Here's the drawing with two shaded views (mm, measured from the low corner). I have some questions. Coordinates: 2 decimals unless noted, no trailing zeros. Loops run counter-clockwise (first coordinate to the right, second up) from the corner with the lowest first, then second, coordinate; pieces in that order, holes last.
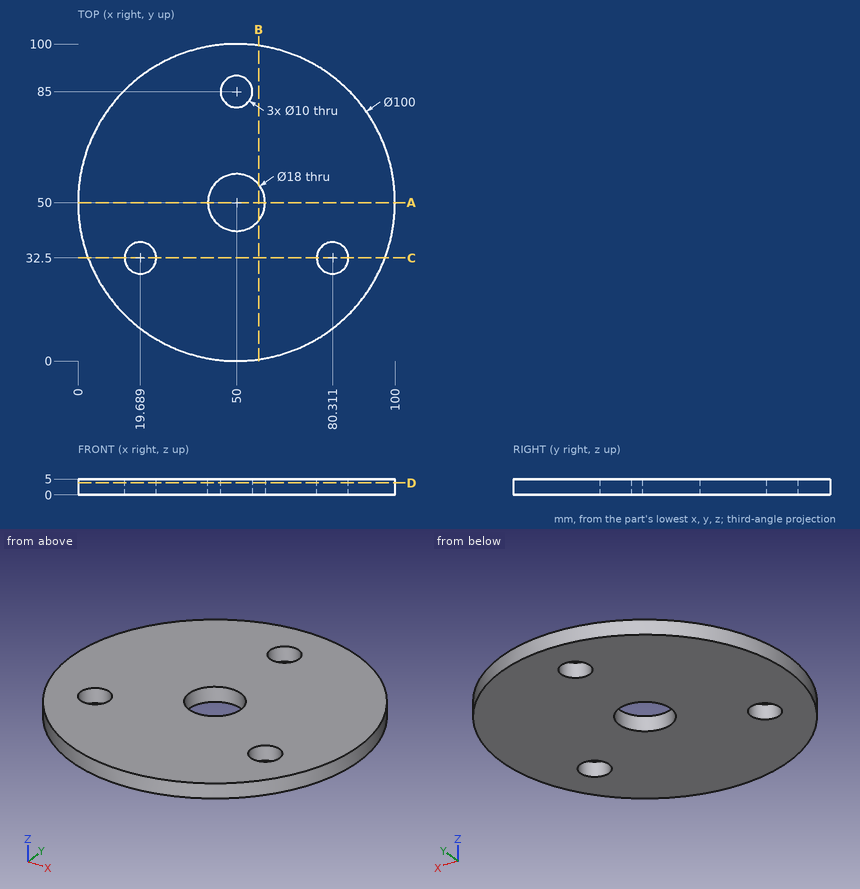
Q1. Suppose I cut it at B-B on x = 57. Write out the boundary of the cut face in (y, z).
Q2. Suppose I cut it at A-A on y = 50. Write out the boundary of the cut face in (x, z), and give its area (3 significant figures).
Q3. Suppose I cut it at D-D on z = 3.75. Write out the boundary of the cut face in (x, y).
Q4. Please list where these lines run through material, in increasing order: probe 1 along Y at (x, z) = (46.5, 4.3); probe 2 along X at (y, z) = (32.5, 1.55); probe 3 along X at (y, z) = (28.5, 3.2).
Q5. Suppose I cut it at C-C on y = 32.5. Write out the boundary of the cut face in (x, z).
Q6. Will these pins go through, and if not, where does the flat tip stop? P1, Ø6, axis at x = 50, y = 85, coming from the -Z side; P2, Ø1.5, axis at x = 13, z = 2, coming from the +Y side; P3, Ø3, axis at x = 79, z = 4.5, coming from the -Y side; P4, Ø3, axis at y = 38, z = 3, coming from the -X side (3 decimals).
Check values:
1. outline: (0.49, 0) - (44.34, 0) - (44.34, 5) - (0.49, 5) - close; (55.66, 0) - (99.51, 0) - (99.51, 5) - (55.66, 5) - close
2. outline: (0, 0) - (41, 0) - (41, 5) - (0, 5) - close; (59, 0) - (100, 0) - (100, 5) - (59, 5) - close
2. area: 410 mm2
3. outline: circle Ø100 at (50, 50); hole circle Ø10 at (19.69, 32.5); hole circle Ø18 at (50, 50); hole circle Ø10 at (50, 85); hole circle Ø10 at (80.31, 32.5)
4. probe 1: y = 0.12 to 41.71, 58.29 to 81.43, 88.57 to 99.88
4. probe 2: x = 3.16 to 14.69, 24.69 to 75.31, 85.31 to 96.84
4. probe 3: x = 4.86 to 16.69, 22.69 to 77.31, 83.31 to 95.14
5. outline: (3.16, 0) - (14.69, 0) - (14.69, 5) - (3.16, 5) - close; (24.69, 0) - (75.31, 0) - (75.31, 5) - (24.69, 5) - close; (85.31, 0) - (96.84, 0) - (96.84, 5) - (85.31, 5) - close
6. P1: passes through
6. P2: stops at y = 84.44
6. P3: stops at y = 8.24
6. P4: stops at x = 1.115
